Geometry check sheet. Reference: the model listing, model coordinates, mm. Coordinates: 2 decimals unless noted, no trailing zeros. Loops run counter-clockwise (first coordinate to the right, second up) from the corner with the lowest first, then second, coordinate; pieces in that order, holes last.
from build123d import *

# Parameters (mm, degrees)
SKETCH1_R               = 3
SKETCH1_R_2             = 2
BOSS_EXTRUDE1_DEPTH     = 350
CUT_EXTRUDE1_DEPTH      = 351.025713341
CUT_EXTRUDE1_DEPTH_BACK = 351.025713341
SKETCH3_R               = 0.75


with BuildPart() as part:
    # Sketch1 → Boss-Extrude1 (new body)
    with BuildSketch(Plane.XY):
        Circle(SKETCH1_R)
        Circle(SKETCH1_R_2, mode=Mode.SUBTRACT)
    extrude(amount=BOSS_EXTRUDE1_DEPTH)

    # Sketch3 → Cut-Extrude1 (cut, two sides: drawn at the far end of the back side and taken through both)
    with BuildSketch(Plane(origin=(0, 0, 0), x_dir=(0, 1, 0), z_dir=(-1, 0, 0)).offset(-CUT_EXTRUDE1_DEPTH_BACK)):
        with Locations(Location((0, -40, 0), (0, 0, 270))):
            Circle(SKETCH3_R)
        with Locations(Location((0, -310, 0), (0, 0, 270))):
            Circle(SKETCH3_R)
    extrude(amount=CUT_EXTRUDE1_DEPTH + CUT_EXTRUDE1_DEPTH_BACK, mode=Mode.SUBTRACT)


solid = part.part
(1) Gauge pin test, flat end, axial feed: pin 1 Ø1 at (x, z) = (-1.5, 88) entering from -Y. Record the tip position at first contact, or that the pin passes through.
Findings:
pin 1: stops at y = -2.83
(2) Sectioned sample at A-A on x = 0. Record the cut outline in (y, z).
Findings:
outline: (-3, 0) - (-2, 0) - (-2, 350) - (-3, 350) - close; (2, 0) - (3, 0) - (3, 350) - (2, 350) - close
(3) Sectioned sample at B-B on z = 323. Record the cut outline in (x, y).
Findings:
outline: circle Ø6 at (0, 0); hole circle Ø4 at (0, 0)
(4) Scan lines: L1, parallel to X at y = 0, z = 143; L2, parallel to X at y = 0.5, z = 277; L3, parallel to Y at x = 2.25, z = 310. Record each from-to range of solid material in increasing order.
Findings:
L1: x = -3 to -2, 2 to 3
L2: x = -2.96 to -1.94, 1.94 to 2.96
L3: y = -1.98 to -0.75, 0.75 to 1.98
